from build123d import *

# Parameters (mm, degrees)
EXTRUDE_1_DEPTH = 110


with BuildPart() as part:
    # 草图1 → 凸台-拉伸1 (new body)
    with BuildSketch(Plane.XY):
        Polygon((0, 0), (0, -60), (-150, -60), (-150, -55), (-5, -55), (-5, 0), align=None)
    extrude(amount=EXTRUDE_1_DEPTH)


solid = part.part
Input: part model. Units: mm. Frame: model coordinates. A direction names the side the tool comes from. Coordinates: 2 decimals unless noted, no trailing zeros. Loops run counter-clockwise (first coordinate to the right, second up) from the corner with the lowest first, then second, coordinate; pieces in that order, holes last.
(1) Material intervals for probe 1 along X at (y, z) = (-36, 103.5); probe 2 along Y at (x, z) = (-63.5, 60.5), sorted ascending.
(2) First-contact query: pin 1 Ø4 at (x, z) = (-34.5, 55.5) entering from +Y; pin 2 Ø16.5 at (y, z) = (-21.5, 49) entering from -X. Flat tips, straight axial feed; report the tip coordinate or a pass-through.
(3) Section C-C on x = -35. Return the cut outline in (y, z).
(4) Section B-B on y = -10. Return the cut outline in (x, z), then the cut area to 3 significant figures.
(5) Set-up query: faces 1 (the face through (-3, 0, 54)), 2 (the face through (-5, -28, 54)). Return all of +Z, -Z, +X, -X, +Y, -Y with unobstructed straight access to the full face (end or side cutting, diameter ignored); none if empty.
(6) Section A-A on z = 52.5. Return the cut outline in (x, y).
Data:
1. probe 1: x = -5 to 0
1. probe 2: y = -60 to -55
2. pin 1: stops at y = -55
2. pin 2: stops at x = -5
3. outline: (-60, 0) - (-55, 0) - (-55, 110) - (-60, 110) - close
4. outline: (-5, 0) - (0, 0) - (0, 110) - (-5, 110) - close
4. area: 550 mm2
5. face 1: +Z, -Z, +X, -X, +Y
5. face 2: +Z, -Z, -X, +Y
6. outline: (-150, -60) - (0, -60) - (0, 0) - (-5, 0) - (-5, -55) - (-150, -55) - close
